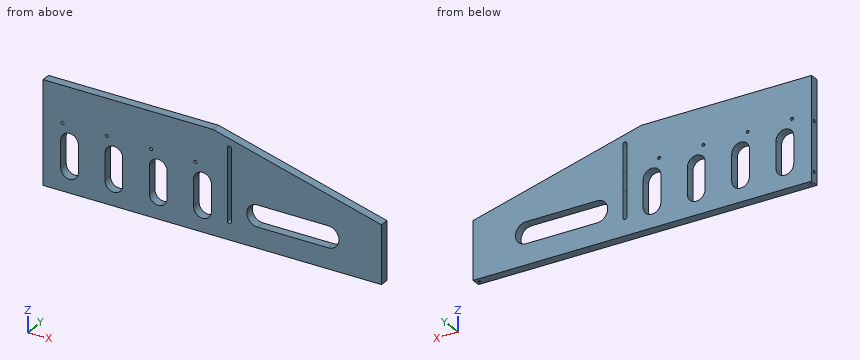
from build123d import *

# Parameters (mm, degrees)
SKETCH_1_W             = 382
SKETCH_1_H             = 80
EXTRUDE_1_DEPTH        = 10
HOLE_WIZARD_M3_1_D     = 2.5
HOLE_WIZARD_M3_1_DEPTH = 8.5
HOLE_WIZARD_M3_1_TIP   = 0.751075774
CUT_EXTRUDE_1_DEPTH    = 196.399590583
PATTERN_LINEAR_1_COUNT = 4
PATTERN_LINEAR_1_PITCH = 50
HOLE_WIZARD_M4_1_D     = 4.5
HOLE_WIZARD_M4_1_2_D   = 3.3
PATTERN_LINEAR_2_COUNT = 4
PATTERN_LINEAR_2_PITCH = 50
HOLE_WIZARD_M4_2_D     = 3.3
HOLE_WIZARD_M4_2_DEPTH = 10.1
HOLE_WIZARD_M4_2_TIP   = 0.991420021
CUT_EXTRUDE_3_DEPTH    = 10
MOVE_FACE_1_BY         = 35
CUT_EXTRUDE_4_DEPTH    = 206.440989094
CHAMFER_1_SIZE         = 190
CHAMFER_1_SIZE2        = 50
CUT_EXTRUDE_2_DEPTH    = 206.440989094


with BuildPart() as part:
    # 草图1 → 凸台-拉伸1 (new body)
    with BuildSketch(Plane(origin=(0, 0, 0), x_dir=(1, 0, 0), z_dir=(0, 1, 0))):
        Rectangle(SKETCH_1_W, SKETCH_1_H)
    extrude(amount=EXTRUDE_1_DEPTH)

    # M3 螺纹孔1
    with Locations(Plane(origin=(0, 0, -40), x_dir=(-1, 0, 0), z_dir=(0, 0, -1))):
        with Locations((187, 5), (-187, 5)):
            Hole(HOLE_WIZARD_M3_1_D / 2, depth=HOLE_WIZARD_M3_1_DEPTH)
            with Locations((0, 0, -(HOLE_WIZARD_M3_1_DEPTH + HOLE_WIZARD_M3_1_TIP / 2))):  # 118° drill point
                Cone(0, HOLE_WIZARD_M3_1_D / 2, HOLE_WIZARD_M3_1_TIP, mode=Mode.SUBTRACT)

    # 草图4 → 切除-拉伸1 (cut, through all)
    with BuildSketch(Plane(origin=(0, 10, 0), x_dir=(1, 0, 0), z_dir=(0, 1, 0))):
        with BuildLine():
            Line((-1, 15), (-1, -15))
            ThreePointArc((-1, -15), (-11, -25), (-21, -15))
            Line((-21, -15), (-21, 15))
            ThreePointArc((-21, 15), (-11, 25), (-1, 15))
        make_face()
    cut_extrude_1 = extrude(amount=-CUT_EXTRUDE_1_DEPTH, mode=Mode.SUBTRACT)

    # 阵列(线性)1: 切除-拉伸1 ×4
    with Locations(*[(-i * PATTERN_LINEAR_1_PITCH, 0, 0) for i in range(1, PATTERN_LINEAR_1_COUNT)]):
        add(cut_extrude_1, mode=Mode.SUBTRACT)

    # Hole Wizard M4 _1 (through all)
    with Locations(Plane(origin=(0, 10, 0), x_dir=(1, 0, 0), z_dir=(0, 1, 0))):
        with Locations((19.5, -11), (19.5, -31)):
            Hole(HOLE_WIZARD_M4_1_D / 2)

    # Hole Wizard M4 _1 2 (through all)
    with Locations(Plane(origin=(0, 10, 0), x_dir=(1, 0, 0), z_dir=(0, 1, 0))):
        with Locations((-19, -34)):
            hole_wizard_m4_1_2 = Hole(HOLE_WIZARD_M4_1_2_D / 2)

    # 阵列(线性)2: Hole Wizard M4 _1 2 ×4
    with Locations(*[(-i * PATTERN_LINEAR_2_PITCH, 0, 0) for i in range(1, PATTERN_LINEAR_2_COUNT)]):
        add(hole_wizard_m4_1_2, mode=Mode.SUBTRACT)

    # M4 螺纹孔2
    with Locations(Plane.ZY.offset(191)):
        with Locations((27.5, 5), (-27.5, 5)):
            Hole(HOLE_WIZARD_M4_2_D / 2, depth=HOLE_WIZARD_M4_2_DEPTH)
            with Locations((0, 0, -(HOLE_WIZARD_M4_2_DEPTH + HOLE_WIZARD_M4_2_TIP / 2))):  # 118° drill point
                Cone(0, HOLE_WIZARD_M4_2_D / 2, HOLE_WIZARD_M4_2_TIP, mode=Mode.SUBTRACT)

    # 草图14 → 切除-拉伸3 (cut)
    with BuildSketch(Plane.XZ):
        with BuildLine():
            Line((21.749999636, 33.25), (21.749999636, 28.75))
            ThreePointArc((21.749999636, 28.75), (19.499999636, 26.5), (17.249999636, 28.75))
            Line((17.249999636, 28.75), (17.249999636, 33.25))
            ThreePointArc((17.249999636, 33.25), (19.499999636, 35.5), (21.749999636, 33.25))
        make_face()
        with BuildLine():
            Line((21.749999636, 13.25), (21.749999636, 8.75))
            ThreePointArc((21.749999636, 8.75), (19.499999636, 6.5), (17.249999636, 8.75))
            Line((17.249999636, 8.75), (17.249999636, 13.25))
            ThreePointArc((17.249999636, 13.25), (19.499999636, 15.5), (21.749999636, 13.25))
        make_face()
    extrude(amount=-CUT_EXTRUDE_3_DEPTH, mode=Mode.SUBTRACT)

    # Move Face 1: a face moved outward by 35.0
    extrude(part.faces().sort_by_distance((0, 5, 40))[0], amount=MOVE_FACE_1_BY, dir=(0, 0, 1))

    # 草图15 → 切除-拉伸4 (cut, through all)
    with BuildSketch(Plane.XZ):
        with BuildLine():
            Line((21.749999636, 60), (21.749999636, -20))
            ThreePointArc((21.749999636, -20), (19.499999636, -22.25), (17.249999636, -20))
            Line((17.249999636, -20), (17.249999636, 60))
            ThreePointArc((17.249999636, 60), (19.499999636, 62.25), (21.749999636, 60))
        make_face()
    extrude(amount=-CUT_EXTRUDE_4_DEPTH, mode=Mode.SUBTRACT)

    # 倒角1
    chamfer_1_edges = [part.edges().sort_by_distance(p)[0] for p in [
        (191, 5, 75),
    ]]
    chamfer_1_side = [part.faces().sort_by_distance(p)[0] for p in [
        (0, 5, 75),
    ]]
    chamfer(chamfer_1_edges, length=CHAMFER_1_SIZE, length2=CHAMFER_1_SIZE2, reference=chamfer_1_side[0])

    # 草图5 → 切除-拉伸2 (cut, through all)
    with BuildSketch(Plane(origin=(0, 10, 0), x_dir=(1, 0, 0), z_dir=(0, 1, 0))):
        with BuildLine():
            Line((131, -7), (51, -7))
            ThreePointArc((51, -7), (39, 5), (51, 17))
            Line((51, 17), (131, 17))
            ThreePointArc((131, 17), (143, 5), (131, -7))
        make_face()
    extrude(amount=-CUT_EXTRUDE_2_DEPTH, mode=Mode.SUBTRACT)


solid = part.part
Build history of the part. All positions in model axes, mm. Round coordinates to 2 decimals unless told otherwise and drop trailing zeros. Order: outer loops, then holes, each group sorted by start corner. A loop starts at its lowest first (then second) coordinate and runs counter-clockwise, first axis right, second up. Notation, with made-up numbers: M 81.25,0 L 117.25,0 A6 ccw 117.25,7 Z; hole C 62.5,87.5 d10. An arc over 180 degrees is marked long. Use CSV: the item, a comma, the result in double quotes. Start each with the question number.
(1) Drill centre lines: probe 1 along X at (y, z) = (5, -36.75); probe 2 along Y at (x, z) = (-184, 27); probe 3 along Z at (x, y) = (-119, 7.75). Where is each one in solid material? Low to high.
(2) Cut at A-A on x = -11. List the corners of the cut face in (y, z), then the cut area to 3 significant figures.
(3) Flat gauge pins, fed straight in: P1, Ø1.5, axis at x = -187, y = 5, coming from the -Z side; P2, Ø3, axis at x = -119, z = 34, coming from the -Y side; P3, Ø10, axis at x = -21, z = 11, coming from the -Y side; P4, Ø3, axis at x = 187, y = 5, coming from the +Z side. Where does each tip first touch, or does it go through?
(4) Cut at B-B on z = 48.5. List the corners of the cut face in (x, y).
(5) Cut at C-C on z = 67.5. List the corners of the cut face in (x, y), then the cut area to 4 significant figures.
Findings:
1,probe 1,"x = -191 to -188.25, -185.75 to 185.75, 188.25 to 191"
1,probe 2,"y = 0 to 3.43, 6.57 to 10"
1,probe 3,"z = -40 to -21, 21 to 32.35, 35.65 to 75"
2,outline,"M 0,-40 L 10,-40 L 10,-25 L 0,-25 Z; M 0,25 L 10,25 L 10,75 L 0,75 Z"
2,area,"650 mm^2"
3,P1,"stops at z = -31.2"
3,P2,"passes through"
3,P3,"stops at y = 0"
3,P4,"stops at z = 26.45"
4,outline,"M -191,0 L 17.25,0 L 17.25,10 L -191,10 Z; M 21.75,0 L 101.7,0 L 101.7,10 L 21.75,10 Z"
5,outline,"M -191,0 L 29.5,0 L 29.5,10 L -191,10 Z"
5,area,"2,205 mm^2"
